```python
from build123d import *

# Parameters (mm, degrees)
PLUNGER_PROFILE_SKETCH_W   = 25
PLUNGER_PROFILE_SKETCH_H   = 7.5
PLUNGER_PROFILE_SKETCH_W_2 = 112
PLUNGER_PROFILE_SKETCH_H_2 = 20


with BuildPart() as part:
    # Plunger Profile Sketch → Plunger Body Revolve (revolve)
    with BuildSketch(Plane.XY, mode=Mode.PRIVATE) as plunger_body_revolve_sk:
        with Locations((-23.33175597, 3.75)):
            Rectangle(PLUNGER_PROFILE_SKETCH_W, PLUNGER_PROFILE_SKETCH_H)
        Polygon((-10.83175597, 7.5), (-10.83175597, 0), (-7.83175597, 0), (-7.83175597, 20), (-10.83175597, 17), align=None)
        with Locations((48.16824403, 10)):
            Rectangle(PLUNGER_PROFILE_SKETCH_W_2, PLUNGER_PROFILE_SKETCH_H_2)
        Polygon((104.16824403, 20), (104.16824403, 0), (114.16824403, 0), (114.16824403, 30), align=None)
        Polygon((114.16824403, 30), (114.16824403, 0), (124.16824403, 0), (124.16824403, 30), (114.16824403, 40), align=None)
    revolve(plunger_body_revolve_sk.sketch.rotate(Axis((-51.8095123, 0, 0), (1, 0, 0)), 90), axis=Axis((-51.8095123, 0, 0), (1, 0, 0)))


solid = part.part
```
Source: CAD feature listing. Evaluate the final solid. Frame: model axes, mm. A direction names the side the tool comes from. Coordinates: 2 decimals unless noted, no trailing zeros. Loops run counter-clockwise (first coordinate to the right, second up) from the corner with the lowest first, then second, coordinate; pieces in that order, holes last. Notation, with made-up numbers: M 16.25,78 L 54.25,78 A19 ccw 54.25,106 Z; hole C 2.25,64.25 d5. An arc over 180 degrees is marked long. Use CSV: the item, a comma, the result in double quotes.
(1) Cut plane D-D on x = -21.5. Return loops of the section in (y, z), and give its area (3 significant figures).
Answers follow:
outline,"C 0,0 d15"
area,"177 mm²"
(2) Cut plane A-A on y = 0. Return loops of the section in (x, z), and give its area (3 significant figures).
Answers follow:
outline,"M -35.83,-7.5 L -10.83,-7.5 L -10.83,-17 L -7.83,-20 L 104.17,-20 L 114.17,-30 L 114.17,-40 L 124.17,-30 L 124.17,30 L 114.17,40 L 114.17,30 L 104.17,20 L -7.83,20 L -10.83,17 L -10.83,7.5 L -35.83,7.5 Z"
area,"6,170 mm²"
(3) Cut plane C-C on x = 54. Return loops of the section in (y, z).
Answers follow:
outline,"C 0,0 d40"
(4) Reachability of faces 1 (the face through (-23.157, -6.324, 4.032)), 2 (the face through (-35.832, 0, 0)) from +Z, -Z, +X, -X, +Y, -Y: full face, straight path, thin tool, end or side. Return the list, or none.
Answers follow:
face 1,"-X"
face 2,"+Z, -Z, -X, +Y, -Y"
(5) Contact query for flat-ended pins moving along their axis: pin 1 (6 mm diameter, centred on x = 54, z = 16.5, fed in from +Y); pin 2 (6 mm diameter, centred on y = -22, z = 24, fed in from -X); pin 3 (1 mm diameter, centred on x = 43, z = -7.5, fed in from -Y) (3 decimals). Output: stop coordinate, or through.
Answers follow:
pin 1,"y = 14.76"
pin 2,"x = 113.73"
pin 3,"y = -18.735"
(6) Line query: line 1 (X direction, y = 6.5, z = 8.5); line 2 (X direction, y = -25.5, z = 9.5); line 3 (Y direction, x = 48.5, z = 0). Output: solid intervals per line, ascending. Write a range as [from, to].
Answers follow:
line 1,"[-10.83, 124.17]"
line 2,"[111.38, 124.17]"
line 3,"[-20, 20]"
